Could you check a few things on this drawing? It's one solid part, dimensions in mm from its lowest x, y, z. A direction names the side the tool comes from. Give positions to 0.01 mm unless a question says otherwise; leave off trailing zeros. Order: outer loops, then holes, each group sorted by start corner. A loop starts at its lowest first (then second) coordinate and runs counter-clockwise, first axis right, second up. Notation, with made-up numbers: (25, -22.5) -> (74, -22.5) arc R10 cw to (74, -14.5) -> close; hole circle Ø5 at (6, -16). An arc over 180 degrees is marked (long way). Answer as a JSON object with one key per item and string values.
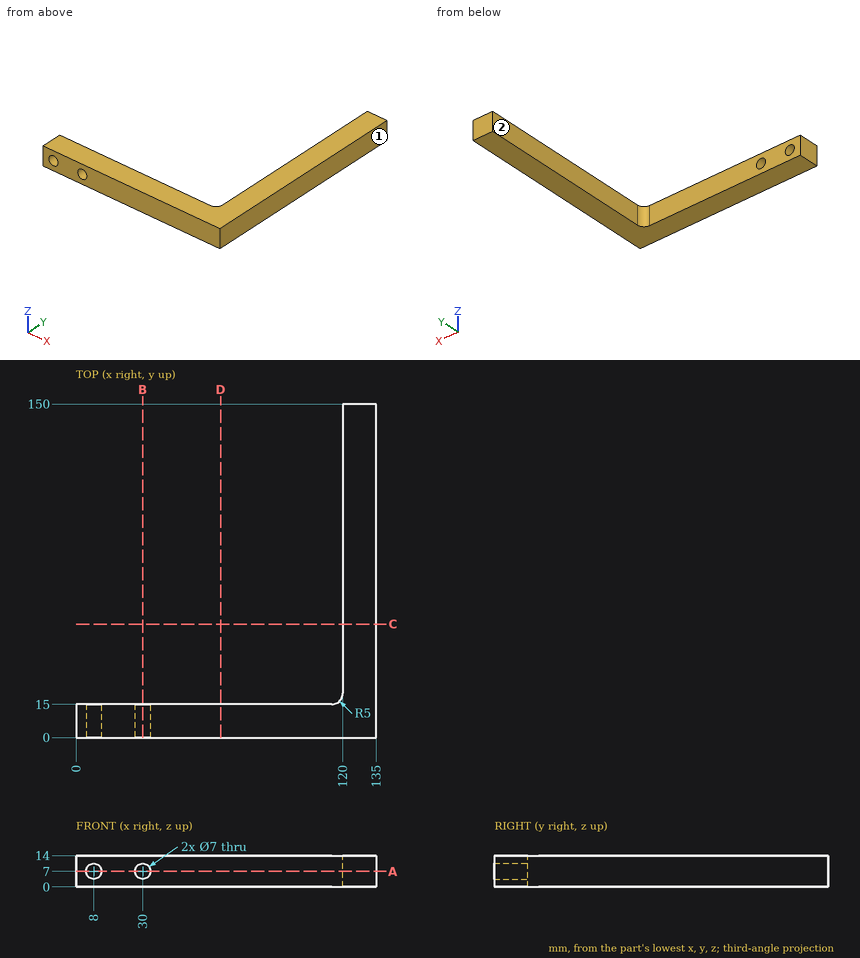
1. If we section it at C-C on y = 51: Please give me the cut outline in (x, z).
Worked answers:
{"outline": "(120, 0) -> (135, 0) -> (135, 14) -> (120, 14) -> close"}
2. Will this pin go through, and if not, where does the flat tip stop? pin 1 Ø8 at (x, z) = (95, 1.5) entering from +Y.
Worked answers:
{"pin 1": "y = 15"}
3. Please list where these lines run through material, in increasing order: L1, parallel to Z at x = 8, y = 4; L2, parallel to Y at x = 41, z = 2.25; L3, parallel to X at y = 129, z = 2.
Worked answers:
{"L1": "0 to 3.5, 10.5 to 14", "L2": "0 to 15", "L3": "120 to 135"}
4. If we section it at D-D on x = 65: Please give me the cut outline in (y, z).
Worked answers:
{"outline": "(0, 0) -> (15, 0) -> (15, 14) -> (0, 14) -> close"}
5. If we section it at A-A on z = 7: Please give me the cut outline in (x, y), then the cut area to 3 significant figures.
Worked answers:
{"outline": "(0, 0) -> (4.5, 0) -> (4.5, 15) -> (0, 15) -> close; (11.5, 0) -> (26.5, 0) -> (26.5, 15) -> (11.5, 15) -> close; (33.5, 0) -> (135, 0) -> (135, 150) -> (120, 150) -> (120, 20) arc R5 cw to (115, 15) -> (33.5, 15) -> close", "area": "3,850 mm²"}
6. For the marked faces 1 and 2, which set-ups out of +Z, -Z, +X, -X, +Y, -Y let a thin tool reach every point of the face, with its end or its side?
Worked answers:
{"face 1": "+Z, -Z, +X, +Y, -Y", "face 2": "+Z, -Z, -X, +Y"}
7. If we section it at B-B on x = 30: Please give me the cut outline in (y, z).
Worked answers:
{"outline": "(0, 0) -> (15, 0) -> (15, 3.5) -> (0, 3.5) -> close; (0, 10.5) -> (15, 10.5) -> (15, 14) -> (0, 14) -> close"}
